Source: CAD feature listing. Evaluate the final solid. Frame: model axes, mm. A direction names the side the tool comes from. Coordinates: 2 decimals unless noted, no trailing zeros. Write each loop counter-clockwise with the first axis right and the second up, starting at its lowest first coordinate (ties: lowest second). Pieces come first, ordered by that corner, then holes. Notation, with made-up numbers: (-14, 21.25) -> (3, 21.25) arc R23 cw to (3, 36.25) -> close; hole circle Ø5 at (11.25, 73.5). An arc over 180 degrees is marked (long way). Write item = value, one per line.
from build123d import *

# Parameters (mm, degrees)
BEARING_HOUSING_SKETCH_R   = 57.5
BEARING_HOUSING_SKETCH_R_2 = 37.5
BEARING_HOUSING_115_DEPTH  = 60
BASE_FOOT_SKETCH_R         = 12.5
BASE_FOOT_DEPTH            = 30
MOUNTING_PAD_SKETCH_R      = 30
MOUNTING_PAD_SKETCH_R_2    = 12.5
MOUNTING_PAD_DEPTH         = 6
SUPPORT_WEB_DEPTH          = 55
SIDE_BOSS_SKETCH_R         = 37.5
SIDE_BOSS_SKETCH_R_2       = 22.5
SIDE_BOSS_75_DEPTH         = 25
GUSSET_RIB_DEPTH           = 13


with BuildPart() as part:
    # Bearing Housing Sketch → Bearing Housing Ø115 (new, symmetric)
    with BuildSketch(Plane(origin=(0, 0, 0), x_dir=(0, 0, -1), z_dir=(1, 0, 0))):
        Circle(BEARING_HOUSING_SKETCH_R)
        Circle(BEARING_HOUSING_SKETCH_R_2, mode=Mode.SUBTRACT)
    extrude(amount=BEARING_HOUSING_115_DEPTH, both=True)



with BuildPart() as body_2:
    # Base Foot Sketch → Base Foot (new body)
    with BuildSketch(Plane(origin=(0, -166, 0), x_dir=(1, 0, 0), z_dir=(0, 1, 0))):
        with BuildLine():
            Line((-60, 111), (60, 111))
            ThreePointArc((60, 111), (96, 75), (60, 39))
            Line((60, 39), (-60, 39))
            ThreePointArc((-60, 39), (-96, 75), (-60, 111))
        make_face()
        with Locations(Location((60, 75, 0), (0, 0, 270))):
            Circle(BASE_FOOT_SKETCH_R, mode=Mode.SUBTRACT)
        with Locations(Location((-60, 75, 0), (0, 0, 270))):
            Circle(BASE_FOOT_SKETCH_R, mode=Mode.SUBTRACT)
    extrude(amount=BASE_FOOT_DEPTH)

    # Mounting Pad Sketch → Mounting Pad (add)
    # profile 1 of 2: a face of its own
    with BuildSketch(Plane(origin=(0, -136, 0), x_dir=(1, 0, 0), z_dir=(0, 1, 0))):
        with Locations(Location((60, 75, 0), (0, 0, 270))):
            Circle(MOUNTING_PAD_SKETCH_R)
        with Locations(Location((60, 75, 0), (0, 0, 270))):
            Circle(MOUNTING_PAD_SKETCH_R_2, mode=Mode.SUBTRACT)
    # profile 2 of 2: a face of its own
    with BuildSketch(Plane(origin=(0, -136, 0), x_dir=(1, 0, 0), z_dir=(0, 1, 0))):
        with Locations(Location((-60, 75, 0), (0, 0, 270))):
            Circle(MOUNTING_PAD_SKETCH_R)
        with Locations(Location((-60, 75, 0), (0, 0, 270))):
            Circle(MOUNTING_PAD_SKETCH_R_2, mode=Mode.SUBTRACT)
    extrude(amount=MOUNTING_PAD_DEPTH)


with BuildPart() as part_1:
    add(part.part)

    add(body_2.part)  # Support Web merges body 2
    # Support Web Sketch → Support Web (add, symmetric)
    with BuildSketch(Plane(origin=(0, 0, 0), x_dir=(0, 0, -1), z_dir=(1, 0, 0))):
        with BuildLine():
            Line((-57.5, 0), (-57.5, -172))
            Line((-57.5, -172), (0, -172))
            Line((0, -172), (0, -166))
            Line((0, -166), (39, -166))
            Line((39, -166), (39, -136))
            Line((39, -136), (-27.5, -136))
            Line((-27.5, -136), (-27.5, -57.5))
            Line((-27.5, -57.5), (0, -57.5))
            ThreePointArc((0, -57.5), (-40.658639918, -40.658639918), (-57.5, 0))
        make_face()
    extrude(amount=SUPPORT_WEB_DEPTH, both=True)



with BuildPart() as body_2_2:
    # Side Boss Sketch → Side Boss Ø75 (new, symmetric)
    with BuildSketch(Plane(origin=(0, 0, 0), x_dir=(0, 0, -1), z_dir=(1, 0, 0))):
        with Locations((-110, -97)):
            Circle(SIDE_BOSS_SKETCH_R)
        with Locations((-110, -97)):
            Circle(SIDE_BOSS_SKETCH_R_2, mode=Mode.SUBTRACT)
    extrude(amount=SIDE_BOSS_75_DEPTH, both=True)


with BuildPart() as part_2:
    add(part_1.part)

    add(body_2_2.part)  # Gusset Rib merges body 2 2
    # Gusset Rib Sketch → Gusset Rib (add, symmetric)
    with BuildSketch(Plane(origin=(0, 0, 0), x_dir=(0, 0, -1), z_dir=(1, 0, 0))):
        with BuildLine():
            Line((-138.406251821, -72.518683502), (-43.556252792, 37.53801863))
            ThreePointArc((-43.556252792, 37.53801863), (-53.901458865, 20.022056144), (-57.5, 0))
            Line((-57.5, 0), (-57.5, -172))
            Line((-57.5, -172), (-129.216934712, -129.201854299))
            ThreePointArc((-129.216934712, -129.201854299), (-72.983281658, -90.998953157), (-138.406251821, -72.518683502))
        make_face()
    extrude(amount=GUSSET_RIB_DEPTH, both=True)


solid = part_2.part
1) Pull-direction query (Y, two-part tool) for faces 1 (the cylindrical face through (0.84, 48.484, -30.912)), 2 (the cylindrical face through (-0.84, 37.18, 4.88)), 3 (the cylindrical face through (72.394, -148.252, -76.627)), 4 (the flat face through (1, -166, -56)); classes: +Y half, -Y half, draft (parallel to the pull), parting line (faces both ways), or undercut.
Answer block:
face_1 = undercut
face_2 = undercut
face_3 = draft
face_4 = -Y half
2) Cut plane D-D, the plane x = 7. Output: boundary loops of the cut face in (y, z).
Answer block:
outline = (-172, 0) -> (-166, 0) -> (-166, -111) -> (-136, -111) -> (-136, 27.5) -> (-57.5, 27.5) -> (-57.5, 0) arc R57.5 ccw (long way) to (37.54, 43.56) -> (-72.52, 138.41) arc R37.5 ccw to (-129.2, 129.22) -> (-172, 57.5) -> close; hole circle Ø45 at (-97, 110); hole circle Ø75 at (0, 0)
3) First-contact query: pin 1 Ø15 at (x, z) = (-60, -75) entering from +Y; pin 2 Ø21 at (x, y) = (-36.5, -90.5) entering from +Z; pin 3 Ø2 at (x, y) = (-55, -73.5) entering from -Z; pin 4 Ø10 at (y, z) = (-44.5, 94.5) entering from +X. Flat tips, straight axial feed; report the tip coordinate or a pass-through.
Answer block:
pin_1 = through
pin_2 = 57.5
pin_3 = 27.5
pin_4 = 13
4) Reachability of faces 5 (the flat face through (-13, -82, 73)), 6 (the flat face through (-60, -130, -62)), 7 (the flat face through (13, -82, 73)), 8 (the flat face through (-34, -85, 57.5)), 9 (the flat face through (-60, -38, 1)) from +Z, -Z, +X, -X, +Y, -Y: full face, straight path, thin tool, end or side. Return the list, or none.
Answer block:
face_5 = -X
face_6 = -Z, +X, -X
face_7 = +X
face_8 = -X, +Y, -Y
face_9 = +Z, -Z, -X, +Y
5) Cut plane B-B, the plane y = -97. Output: boundary loops of the cut face in (x, z), and give its area (3 significant figures).
Answer block:
outline = (-55, 27.5) -> (55, 27.5) -> (55, 57.5) -> (13, 57.5) -> (13, 72.5) -> (25, 72.5) -> (25, 87.5) -> (-25, 87.5) -> (-25, 72.5) -> (-13, 72.5) -> (-13, 57.5) -> (-55, 57.5) -> close; (-25, 132.5) -> (25, 132.5) -> (25, 147.5) -> (-25, 147.5) -> close
area = 5,190 mm2
6) Cut plane C-C, the plane z = 110. Output: boundary loops of the cut face in (x, y), and give its area (3 significant figures).
Answer block:
outline = (-25, -134.5) -> (-13, -134.5) -> (-13, -140.67) -> (13, -140.67) -> (13, -134.5) -> (25, -134.5) -> (25, -119.5) -> (-25, -119.5) -> close; (-25, -74.5) -> (25, -74.5) -> (25, -59.5) -> (13, -59.5) -> (13, -39.56) -> (-13, -39.56) -> (-13, -59.5) -> (-25, -59.5) -> close
area = 2,180 mm2
7) Material intervals for probe 1 along X at (y, z) = (-144, -75); probe 2 along Y at (x, z) = (-14, 2); probe 3 along Y at (x, z) = (-22, -5.5), sorted ascending. Write a range as [from, to].
Answer block:
probe_1 = [-96, -72.5], [-47.5, 47.5], [72.5, 96]
probe_2 = [-172, -136], [-57.5, -37.45], [37.45, 57.47]
probe_3 = [-166, -136], [-57.24, -37.09], [37.09, 57.24]
8) Cut plane A-A, the plane x = 42. Output: boundary loops of the cut face in (y, z), and give its area (3 significant figures).
Answer block:
outline = (-172, 0) -> (-166, 0) -> (-166, -111) -> (-136, -111) -> (-136, -99) -> (-130, -99) -> (-130, -51) -> (-136, -51) -> (-136, 27.5) -> (-57.5, 27.5) -> (-57.5, 0) arc R57.5 ccw (long way) to (0, 57.5) -> (-172, 57.5) -> close; hole circle Ø75 at (0, 0)
area = 14,700 mm2
